```python
from build123d import *

# Parameters (mm, degrees)
SKETCH1_W           = 190
SKETCH1_H           = 16
BOSS_EXTRUDE1_DEPTH = 3.5
HOLE1_D             = 6
HOLE1_DEPTH         = 20
HOLE1_CSINK_D       = 10
HOLE1_CSINK_ANGLE   = 90
CHAMFER1_SIZE       = 1


with BuildPart() as part:
    # Sketch1 → Boss-Extrude1 (new, symmetric)
    with BuildSketch(Plane(origin=(0, 0, 0), x_dir=(1, 0, 0), z_dir=(0, 1, 0))):
        Rectangle(SKETCH1_W, SKETCH1_H)
    extrude(amount=BOSS_EXTRUDE1_DEPTH, both=True)

    # Hole1
    with Locations(Plane(origin=(0, 3.5, 0), x_dir=(1, 0, 0), z_dir=(0, 1, 0))):
        with Locations((-65, 0), (0, 0), (65, 0)):
            CounterSinkHole(HOLE1_D / 2, HOLE1_CSINK_D / 2, depth=HOLE1_DEPTH, counter_sink_angle=HOLE1_CSINK_ANGLE)

    # Chamfer1
    chamfer1_edges = [part.edges().sort_by_distance(p)[0] for p in [
        (0, 3.5, 8),
        (0, -3.5, 8),
        (0, -3.5, -8),
        (95, 0, 8),
        (-95, 0, 8),
        (-95, 0, -8),
        (95, 0, -8),
        (0, 3.5, -8),
    ]]
    chamfer(chamfer1_edges, length=CHAMFER1_SIZE)


solid = part.part
```
Part model, mm, in its own coordinate system. Round coordinates to 2 decimals unless told otherwise and drop trailing zeros. Write each loop counter-clockwise with the first axis right and the second up, starting at its lowest first coordinate (ties: lowest second). Pieces come first, ordered by that corner, then holes. Notation, with made-up numbers: M 71,67.5 L 129,67.5 A29 ccw 129,103.5 Z; hole C -8.75,19.25 d7. An arc over 180 degrees is marked long. Answer as CSV lines item,"result". Start each with the question number.
1) Drill centre lines: L1, parallel to Z at x = 0, y = -0.3; L2, parallel to X at y = 2.25, z = -2; L3, parallel to X at y = 0.25, z = -0.75. Where is each one in solid material? Low to high.
2) Band-saw the part on C-C (x = -56). List the corners of the cut face in (y, z), then the cut area to 3 significant figures.
3) Mould opens along X. For faces 1 (the face through (-1, 3.5, 6)), 2 (the face through (67.4, -1, 1.8)), 3 (the face through (-95, 0, 0)), 4 (the face through (-62, -1, 0)) say: +X half, -X half, draft (parallel to the pull), parting line (faces both ways), or undercut.
4) Drop flat-ended pins along their axis: pin 1 (5 mm diameter, centred on x = 65, z = 0, fed in from +Y); pin 2 (7 mm diameter, centred on x = 0, z = 0, fed in from +Y). Give the stop position or say it passes through.
5) Band-saw the part on B-B (x = 65). List the corners of the cut face in (y, z).
6) Band-saw the part on A-A (z = 0). List the corners of the cut face in (x, y), then the cut area to 3 significant figures.
Worked out:
1,L1,"-8 to -3, 3 to 8"
1,L2,"-95 to -68.17, -61.83 to -3.17, 3.17 to 61.83, 68.17 to 95"
1,L3,"-95 to -67.9, -62.1 to -2.9, 2.9 to 62.1, 67.9 to 95"
2,outline,"M -3.5,-7 L -2.5,-8 L 2.5,-8 L 3.5,-7 L 3.5,7 L 2.5,8 L -2.5,8 L -3.5,7 Z"
2,area,"110 mm²"
3,face 1,"draft"
3,face 2,"undercut"
3,face 3,"-X half"
3,face 4,"undercut"
4,pin 1,"through"
4,pin 2,"y = 2"
5,outline,"M -3.5,-7 L -2.5,-8 L 2.5,-8 L 3.5,-7 L 3.5,-5 L 1.5,-3 L -3.5,-3 Z; M -3.5,3 L 1.5,3 L 3.5,5 L 3.5,7 L 2.5,8 L -2.5,8 L -3.5,7 Z"
6,outline,"M -95,-3.5 L -68,-3.5 L -68,1.5 L -70,3.5 L -95,3.5 Z; M -62,-3.5 L -3,-3.5 L -3,1.5 L -5,3.5 L -60,3.5 L -62,1.5 Z; M 3,-3.5 L 62,-3.5 L 62,1.5 L 60,3.5 L 5,3.5 L 3,1.5 Z; M 68,-3.5 L 95,-3.5 L 95,3.5 L 70,3.5 L 68,1.5 Z"
6,area,"1,190 mm²"
